from build123d import *

# Parameters (mm, degrees)
SKETCH1_R           = 2
BOSS_EXTRUDE1_DEPTH = 17.5
CHAMFER1_SIZE       = 0.5
SKETCH2_W           = 1
SKETCH2_H           = 23
CUT_EXTRUDE1_DEPTH  = 5


with BuildPart() as part:
    # Sketch1 → Boss-Extrude1 (new, symmetric)
    with BuildSketch(Plane.XY):
        Circle(SKETCH1_R)
    extrude(amount=BOSS_EXTRUDE1_DEPTH, both=True)

    # Chamfer1
    chamfer1_edges = [part.edges().sort_by_distance(p)[0] for p in [
        (-2, 0, -17.5),
        (-2, 0, 17.5),
    ]]
    chamfer(chamfer1_edges, length=CHAMFER1_SIZE)

    # Sketch2 → Cut-Extrude1 (cut, symmetric)
    with BuildSketch(Plane(origin=(0, 0, 0), x_dir=(1, 0, 0), z_dir=(0, 1, 0))):
        with Locations((2, 0)):
            Rectangle(SKETCH2_W, SKETCH2_H)
    extrude(amount=CUT_EXTRUDE1_DEPTH, both=True, mode=Mode.SUBTRACT)


solid = part.part
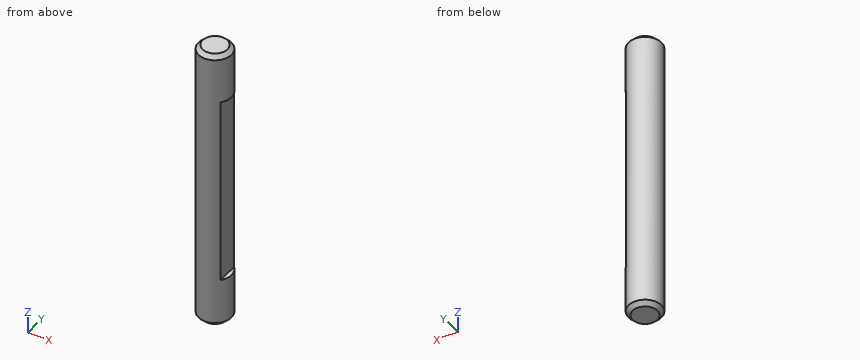
Design review of the part built by this model. Coordinates are the model's own, in mm. Round coordinates to 2 decimals unless told otherwise and drop trailing zeros. Order: outer loops, then holes, each group sorted by start corner. A loop starts at its lowest first (then second) coordinate and runs counter-clockwise, first axis right, second up. Notation, with made-up numbers: M -9,-28.5 L 13,-28.5 A11 cw 13,-13.5 Z; hole C 88.25,-9.5 d2. An arc over 180 degrees is marked long. Answer as CSV lines item,"result". Start each with the question number.
1) Add section A-A (y = 0). Give the boundary of the cut face in (x, z).
2) Wall thickness on line 1 along Z through (x, y) = (1.75, -0.35); line 2 along X through (y, z) = (1.5, 10); line 3 along Z through (x, y) = (0.95, -1.35): over which ranges is each line inside the solid? List them lowest first. Write a range as [from, to].
3) Add section B-B (z = 10). Give the boundary of the cut face in (x, y).
4) For pin 1 Ø1 at (y, z) = (1.5, 9.5) entering from -X, flat-tipped, find the tip position at first contact; note if it passes through.
Resolved:
1,outline,"M -2,-17 L -1.5,-17.5 L 1.5,-17.5 L 2,-17 L 2,-11.5 L 1.5,-11.5 L 1.5,11.5 L 2,11.5 L 2,17 L 1.5,17.5 L -1.5,17.5 L -2,17 Z"
2,line 1,"[-17.22, -11.5], [11.5, 17.22]"
2,line 2,"[-1.32, 1.32]"
2,line 3,"[-17.35, 17.35]"
3,outline,"M 1.5,-1.32 L 1.5,1.32 A2 ccw long Z"
4,pin 1,"x = -1.73"
